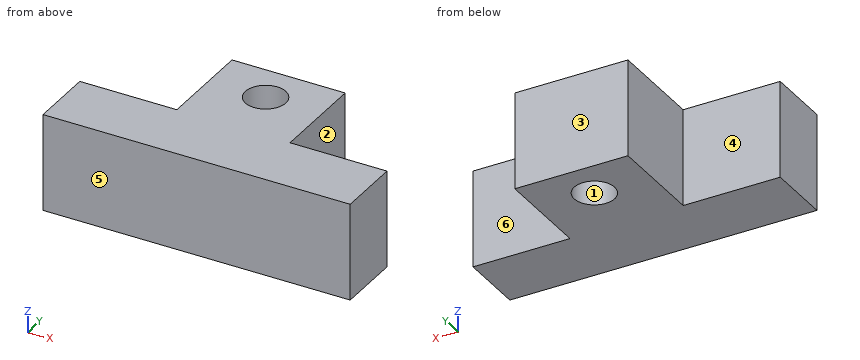
from build123d import *

# Parameters (mm, degrees)
EXTRUDE_1_DEPTH    = 6
HOLE_WIZARD_M6_1_D = 5


with BuildPart() as part:
    # 草图1 → 凸台-拉伸1 (new, symmetric)
    with BuildSketch(Plane.XY):
        Polygon((0, 0), (-7, 0), (-7, -12), (-19, -12), (-19, -20), (19, -20), (19, -12), (7, -12), (7, 0), align=None)
    extrude(amount=EXTRUDE_1_DEPTH, both=True)

    # M6 螺纹孔1 (through all)
    with Locations(Plane(origin=(0, -5, 6), x_dir=(1, 0, 0), z_dir=(0, 0, 1))):
        with Locations((0, 0)):
            Hole(HOLE_WIZARD_M6_1_D / 2)


solid = part.part
Part model, mm, in its own coordinate system. Face numbers are marked on the shaded views. A direction names the side the tool comes from. Coordinates: 2 decimals unless noted, no trailing zeros. Loops run counter-clockwise (first coordinate to the right, second up) from the corner with the lowest first, then second, coordinate; pieces in that order, holes last. Notation, with made-up numbers: M 8,52.25 L 55,52.25 A26 cw 55,80.25 Z; hole C 75.5,25.25 d4. An arc over 180 degrees is marked long. Use a Markdown table: item, result. Add a question column.
Q1. Probe L1, parallel to Y at x = 0, z = -1.5; L2, parallel to Y at x = -12.5, z = -2.75; L3, parallel to X at y = -4.5, z = 0. List the from-to ranges inside material, lowest first.
Q2. Cut at C-C (x = -8). Write the cut outline in (y, z), and give its area (3 significant figures).
Q3. Mould opens along Y. For the marked faces 1, 2 and 3 say: +Y half, -Y half, draft (parallel to the pull), parting line (faces both ways), or undercut.
Q4. Cut at B-B (x = 0). Write the cut outline in (y, z).
Q5. Which spindle directions (+Z, -Z, +X, -X, +Y, -Y) get a long thin tool onto all of the face, cutting with end or side? Do the marked faces 4, 5 and 6. Say none if no direction does.
Q6. Cut at A-A (z = 5). Write the cut outline in (x, y).
Q7. Pin check, flat tips, straight feed: P1, Ø6, axis at x = 11, z = -1, coming from the +Y side; P2, Ø4.5, axis at x = 0, y = -5, coming from the -Z side; P3, Ø1.5, axis at y = -5, z = 3.5, coming from the -X side; P4, Ø6, axis at y = -4.5, z = -2, coming from the +X side. Stop position of each tip, or through.
Worked out:
| question | item | result |
|---|---|---|
| 1 | L1 | y = -20 to -7.5, -2.5 to 0 |
| 1 | L2 | y = -20 to -12 |
| 1 | L3 | x = -7 to -2.45, 2.45 to 7 |
| 2 | outline | M -20,-6 L -12,-6 L -12,6 L -20,6 Z |
| 2 | area | 96.0 mm2 |
| 3 | face 1 | undercut |
| 3 | face 2 | draft |
| 3 | face 3 | +Y half |
| 4 | outline | M -20,-6 L -7.5,-6 L -7.5,6 L -20,6 Z; M -2.5,-6 L 0,-6 L 0,6 L -2.5,6 Z |
| 5 | face 4 | +Z, -Z, -X, +Y |
| 5 | face 5 | +Z, -Z, +X, -X, -Y |
| 5 | face 6 | +Z, -Z, +X, +Y |
| 6 | outline | M -19,-20 L 19,-20 L 19,-12 L 7,-12 L 7,0 L -7,0 L -7,-12 L -19,-12 Z; hole C 0,-5 d5 |
| 7 | P1 | stops at y = -12 |
| 7 | P2 | passes through |
| 7 | P3 | stops at x = -7 |
| 7 | P4 | stops at x = 7 |
